Verification items for the finished model (mm, model axes). Give positions to 0.01 mm unless a question says otherwise; leave off trailing zeros. Loops run counter-clockwise (first coordinate to the right, second up) from the corner with the lowest first, then second, coordinate; pieces in that order, holes last. Notation, with made-up numbers: M 9,18 L 44,18 A21 ccw 44,56 Z; hole C 6.25,49.25 d5. An arc over 180 degrees is marked long. Use CSV: the item, a comma, the result in double quotes.
from build123d import *

# Parameters (mm, degrees)
SKETCH1_R           = 2.75
BOSS_EXTRUDE1_DEPTH = 3
SKETCH2_W           = 6
SKETCH2_H           = 6
BOSS_EXTRUDE2_DEPTH = 1.5


with BuildPart() as part:
    # Sketch1 → Boss-Extrude1 (new body)
    with BuildSketch(Plane(origin=(0, 0, 0), x_dir=(1, 0, 0), z_dir=(0, 1, 0))):
        with Locations(Location((0, 0, 0), (0, 0, 270))):
            Circle(SKETCH1_R)
    extrude(amount=BOSS_EXTRUDE1_DEPTH)

    # Sketch2 → Boss-Extrude2 (add)
    with BuildSketch(Plane.XZ):
        Rectangle(SKETCH2_W, SKETCH2_H)
    extrude(amount=BOSS_EXTRUDE2_DEPTH)


solid = part.part
(1) Mould release check, pull along Y, two halves, no side actions. Record for faces 1 (the flat face through (0, -1.5, 0)), 2 (the cylindrical face through (-2.685, 1.479, -0.596)), 3 (the flat face through (0, 3, 0)): released by +Y, released by -Y, zero draft, split by the parting line, or undercut.
Calculated:
face 1,"released by -Y"
face 2,"zero draft"
face 3,"released by +Y"
(2) Section check B-B on z = 0. Record the cut outline in (x, y), plus the area to 3 significant figures.
Calculated:
outline,"M -3,-1.5 L 3,-1.5 L 3,0 L 2.75,0 L 2.75,3 L -2.75,3 L -2.75,0 L -3,0 Z"
area,"25.5 mm²"
(3) Section check C-C on y = 2.3. Record the cut outline in (x, z).
Calculated:
outline,"C 0,0 d5.5"
(4) Section check A-A on x = 0. Record the cut outline in (y, z), plus the area to 3 significant figures.
Calculated:
outline,"M -1.5,-3 L 0,-3 L 0,-2.75 L 3,-2.75 L 3,2.75 L 0,2.75 L 0,3 L -1.5,3 Z"
area,"25.5 mm²"
(5) Depth check by flat-ended pin: pin 1 Ø2 at (y, z) = (2, -2) entering from +X. Enter the tip coordinate at first touch or a pass-through.
Calculated:
pin 1,"stops at x = 2.56"
(6) Scan lines: L1, parallel to Y at x = -2, z = -2.4; L2, parallel to X at y = 0.8, z = -2.5; L3, parallel to Z at x = 0.25, y = 0.4. Record each from-to range of solid material in increasing order. Write a range as from..to.
Calculated:
L1,"y = -1.5..0"
L2,"x = -1.15..1.15"
L3,"z = -2.74..2.74"
